```python
from build123d import *

# Parameters (mm, degrees)
BOSS_EXTRUDE1_DEPTH        = 12
F_6_5_6_5_DIAMETER_HOLE1_D = 6.5
CHAMFER1_SIZE              = 2


with BuildPart() as part:
    # Sketch1 → Boss-Extrude1 (new body)
    with BuildSketch(Plane(origin=(0, 6, 0), x_dir=(1, 0, 0), z_dir=(0, 1, 0))):
        Polygon((-20, -5), (25, -5), (25, 5), (-25, 5), (-25, 0), align=None)
    extrude(amount=-BOSS_EXTRUDE1_DEPTH)

    # Ø6.5 (6.5) Diameter Hole1 (through all)
    with Locations(Plane.XY.offset(5)):
        with Locations((13, 0)):
            Hole(F_6_5_6_5_DIAMETER_HOLE1_D / 2)

    # Chamfer1
    chamfer1_edges = [part.edges().sort_by_distance(p)[0] for p in [
        (25, 0, 5),
    ]]
    chamfer(chamfer1_edges, length=CHAMFER1_SIZE)


solid = part.part
```
Check sheet for the modelled part. Datum: model origin and axes. Units: mm. Round coordinates to 2 decimals unless told otherwise and drop trailing zeros. Loops run counter-clockwise (first coordinate to the right, second up) from the corner with the lowest first, then second, coordinate; pieces in that order, holes last. Notation, with made-up numbers: (-2, -24) -> (10, -24) arc R28 cw to (10, -2) -> close; hole circle Ø9 at (14.25, 31.5). An arc over 180 degrees is marked (long way). Answer in a Markdown table with one row per item.
Q1. Sectioned sample at B-B on z = 1.5. Enter the section's corners in (x, y).
Data:
| item | result |
|---|---|
| outline | (-23.5, -6) -> (25, -6) -> (25, 6) -> (-23.5, 6) -> close; hole circle Ø6.5 at (13, 0) |
Q2. Sectioned sample at C-C on x = 13. Enter the section's corners in (y, z), then the cut area to 3 significant figures.
Data:
| item | result |
|---|---|
| outline | (-6, -5) -> (-3.25, -5) -> (-3.25, 5) -> (-6, 5) -> close; (3.25, -5) -> (6, -5) -> (6, 5) -> (3.25, 5) -> close |
| area | 55.0 mm^2 |
Q3. Thickness scan on L1, parallel to Y at x = 13, z = -2; L2, parallel to Y at x = 15.5, z = 0; L3, parallel to X at y = 1, z = 2. Record the ranges inside material, lowest first.
Data:
| item | result |
|---|---|
| L1 | y = -6 to -3.25, 3.25 to 6 |
| L2 | y = -6 to -2.08, 2.08 to 6 |
| L3 | x = -23 to 9.91, 16.09 to 25 |
Q4. Sectioned sample at A-A on y = 0. Enter the section's corners in (x, z), then the cut area to 4 significant figures.
Data:
| item | result |
|---|---|
| outline | (-25, -5) -> (9.75, -5) -> (9.75, 5) -> (-20, 5) -> (-25, 0) -> close; (16.25, -5) -> (25, -5) -> (25, 3) -> (23, 5) -> (16.25, 5) -> close |
| area | 420.5 mm^2 |
Q5. Sectioned sample at D-D on x = -21.5. Enter the section's corners in (y, z).
Data:
| item | result |
|---|---|
| outline | (-6, -5) -> (6, -5) -> (6, 3.5) -> (-6, 3.5) -> close |
Q6. Release check for a two-part mould opening along X. For faces 1 (the face through (0, 6, 0)), 2 (the face through (16.247, 0.143, -0.07)), 3 (the face through (-23, 0, 2)) record: released by +X, released by -X, zero draft, split by the parting line, or undercut.
Data:
| item | result |
|---|---|
| face 1 | zero draft |
| face 2 | undercut |
| face 3 | released by -X |
